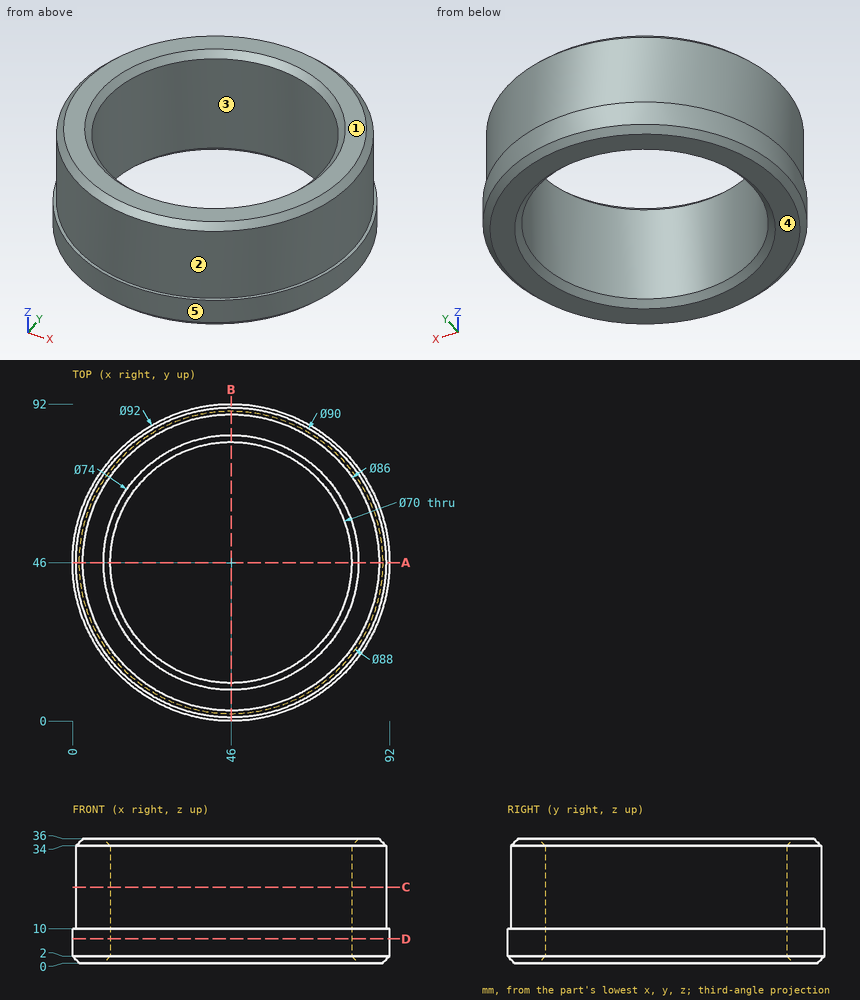
Source: three-view drawing plus pictorial views. Frame: mm from the lowest corner of the part. A direction names the side the tool comes from. Give positions to 0.01 mm unless a question says otherwise; leave off trailing zeros. Order: outer loops, then holes, each group sorted by start corner. A loop starts at its lowest first (then second) coordinate and runs counter-clockwise, first axis right, second up. Notation, with made-up numbers: (17.5, 47) - (59.5, 47) arc R20 ccw to (59.5, 69) - close; hole circle Ø11 at (67, -12.75). An arc over 180 degrees is marked (long way). Answer as a JSON object with one key per item and string values. Group by question number.
Q1. Cut plane D-D, the plane z = 7. Output: boundary loops of the cut face in (x, y), then the cut area to 3 significant figures.
Q2. Cut plane A-A, the plane y = 46. Output: boundary loops of the cut face in (x, z), then the cut area to 3 significant figures.
Q3. Mould query, pull axis X, two halves, no side actions, for the marked faces 3, 4 and 5. Classes: pulls with the +X half, pulls with the -X half, needs draft (parallel to the pull), parting line crosses it, or undercut.
Q4. Line query: probe 1 along Y at (x, z) = (32, 16.5); probe 2 along Y at (x, z) = (46, 9.5); probe 3 along X at (y, z) = (57, 21). Output: solid intervals per line, ascending.
Q5. Set-up query: the marked faces 1 and 2. Return all of +Z, -Z, +X, -X, +Y, -Y with unobstructed straight access to the full face (end or side cutting, diameter ignored); none if empty.
Q6. First-contact query: pin 1 Ø4 at (y, z) = (75.5, 13) entering from -X; pin 2 Ø8 at (y, z) = (16, 27) entering from +X; pin 3 Ø4 at (x, y) = (17, 12) entering from +Z; pin 4 Ø1.5 at (x, z) = (34, 12.5) entering from -Y. Flat tips, straight axial feed; report the tip coordinate or a pass-through.
Q7. Cut plane C-C, the plane z = 22. Output: boundary loops of the cut face in (x, y), then the cut area to 3 significant figures.
Results:
{
 "1": {"outline": "circle Ø92 at (46, 46); hole circle Ø70 at (46, 46)", "area": "2,800 mm^2"},
 "2": {"outline": "(0, 2) - (2, 0) - (9, 0) - (11, 2) - (11, 34) - (9, 36) - (3, 36) - (1, 34) - (1, 10) - (0, 10) - close; (81, 2) - (83, 0) - (90, 0) - (92, 2) - (92, 10) - (91, 10) - (91, 34) - (89, 36) - (83, 36) - (81, 34) - close", "area": "724 mm^2"},
 "3": {"face 3": "undercut", "face 4": "needs draft", "face 5": "parting line crosses it"},
 "4": {"probe 1": "3.23 to 13.92, 78.08 to 88.77", "probe 2": "0 to 11, 81 to 92", "probe 3": "2.37 to 12.77, 79.23 to 89.63"},
 "5": {"face 1": "+Z, +X, -X, +Y, -Y", "face 2": "+Z"},
 "6": {"pin 1": "x = 10.38", "pin 2": "x = 82.73", "pin 3": "z = 36", "pin 4": "y = 2.43"},
 "7": {"outline": "circle Ø90 at (46, 46); hole circle Ø70 at (46, 46)", "area": "2,510 mm^2"}
}
